Verification items for the finished model (mm, model axes). Face numbers are marked on the shaded views. A direction names the side the tool comes from. Give positions to 0.01 mm unless a question says otherwise; leave off trailing zeros. Write each loop counter-clockwise with the first axis right and the second up, starting at its lowest first coordinate (ties: lowest second). Pieces come first, ordered by that corner, then holes. Notation, with made-up numbers: (12.5, 86.5) - (17.5, 86.5) arc R12 cw to (17.5, 96.5) - close; hole circle Ø7 at (-23, 7). An arc over 180 degrees is marked (long way). Answer as a JSON object with one key per item and string values. Group by question number.
Item 1: Sectioned sample at D-D, the plane z = 9.25. Record the boundary of the cut face in (x, y), and give its area (3 significant figures).
Item 2: Scan lines: line 1 along X through (y, z) = (-12, 6); line 2 along Y through (x, z) = (10, 2.5); line 3 along Z through (x, y) = (0, 6). Record each from-to range of solid material in increasing order. Write a range as [from, to].
Item 3: Sectioned sample at A-A, the plane z = 2.5. Record the boundary of the cut face in (x, y).
Item 4: Go/stop test with flat-tipped pins: pin 1 (5.5 mm diameter, centred on x = -7.5, y = 5.5, fed in from -Z); pin 2 (6.5 mm diameter, centred on x = -10, y = -10, fed in from +Z); pin 3 (1.5 mm diameter, centred on x = -7, z = 8, fed in from +Y); pin 4 (16 mm diameter, centred on x = -10, y = -10, fed in from +Z). Record where each tip stops, or that it passes through.
Item 5: Tool access check on the marked faces 4, 5 and 6. Record the directions out of +Z, -Z, +X, -X, +Y, -Y that give a thin tool (end or side, any length) a straight path to the whole face; none if there is none.
Item 6: Sectioned sample at B-B, the plane y = -10. Record the boundary of the cut face in (x, z), and give its area (3 significant figures).
Item 7: Draft check along X on the marked faces 1, 2 and 3. Enter one of: +X half, -X half, draft (parallel to the pull), parting line (faces both ways), or undercut.
Item 8: Sectioned sample at C-C, the plane x = -6.5. Record the boundary of the cut face in (y, z), and give its area (3 significant figures).
```python
from build123d import *

# Parameters (mm, degrees)
SKETCH_1_W                   = 35
SKETCH_1_H                   = 35
EXTRUDE_1_DEPTH              = 20
CHAMFER_1_SIZE               = 2
M12X1_25_1_D                 = 10.5
HOLE_WIZARD_M8_1_D           = 6.8
HOLE_WIZARD_M5_1_D           = 5.5
HOLE_WIZARD_M5_1_CBORE_D     = 10
HOLE_WIZARD_M5_1_CBORE_DEPTH = 12
SKETCH_11_W                  = 10
SKETCH_11_H                  = 22
CUT_EXTRUDE_1_DEPTH          = 44.945989578


with BuildPart() as part:
    # 草图1 → 凸台-拉伸1 (new body)
    with BuildSketch(Plane.XY):
        Rectangle(SKETCH_1_W, SKETCH_1_H)
    extrude(amount=EXTRUDE_1_DEPTH)

    # 倒角1
    chamfer_1_edges = [part.edges().sort_by_distance(p)[0] for p in [
        (17.5, -17.5, 10),
        (-17.5, -17.5, 10),
        (-17.5, 17.5, 10),
        (17.5, 17.5, 10),
    ]]
    chamfer(chamfer_1_edges, length=CHAMFER_1_SIZE)

    # M12x1.25 螺纹孔1 (through all)
    with Locations(Plane.XY.offset(20)):
        with Locations((7.5, 5.5)):
            Hole(M12X1_25_1_D / 2)

    # M8 螺纹孔1 (through all)
    with Locations(Plane.XY.offset(20)):
        with Locations((-7.5, 5.5)):
            Hole(HOLE_WIZARD_M8_1_D / 2)

    # M5 六角圆柱头螺钉的柱形沉头孔1 (through all)
    with Locations(Plane.XY.offset(20)):
        with Locations((-10, -10), (10, -10)):
            CounterBoreHole(HOLE_WIZARD_M5_1_D / 2, HOLE_WIZARD_M5_1_CBORE_D / 2, HOLE_WIZARD_M5_1_CBORE_DEPTH)

    # 草图11 → 切除-拉伸1 (cut, through all)
    with BuildSketch(Plane(origin=(17.5, 0, 0), x_dir=(0, 0, -1), z_dir=(1, 0, 0))):
        with Locations((-5, 6.5)):
            Rectangle(SKETCH_11_W, SKETCH_11_H)
    extrude(amount=-CUT_EXTRUDE_1_DEPTH, mode=Mode.SUBTRACT)


solid = part.part
```
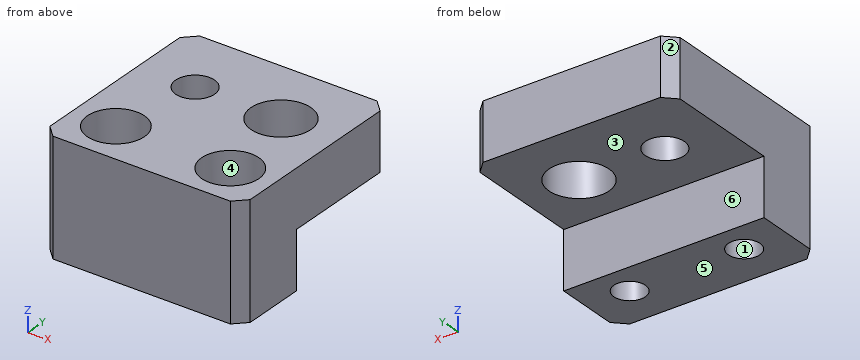
Geometry check:
{
 "1": {"outline": "(-17.5, -15.5) - (-15.5, -17.5) - (15.5, -17.5) - (17.5, -15.5) - (17.5, -4.5) - (-17.5, -4.5) - close; hole circle Ø10 at (-10, -10); hole circle Ø10 at (10, -10)", "area": "294 mm^2"},
 "2": {"line 1": "[-17.5, -11.89], [-8.11, 8.11], [11.89, 17.5]", "line 2": "[-17.5, -12.75], [-7.25, -4.5]", "line 3": "[10, 20]"},
 "3": {"outline": "(-17.5, -15.5) - (-15.5, -17.5) - (15.5, -17.5) - (17.5, -15.5) - (17.5, -4.5) - (-17.5, -4.5) - close; hole circle Ø5.5 at (-10, -10); hole circle Ø5.5 at (10, -10)"},
 "4": {"pin 1": "through", "pin 2": "z = 8", "pin 3": "y = -4.5", "pin 4": "z = 20"},
 "5": {"face 4": "+Z", "face 5": "-Z, +X, -X, +Y, -Y", "face 6": "-Z, +X, -X, +Y"},
 "6": {"outline": "(-17.5, 0) - (-12.75, 0) - (-12.75, 8) - (-15, 8) - (-15, 20) - (-17.5, 20) - close; (-7.25, 0) - (7.25, 0) - (7.25, 8) - (5, 8) - (5, 20) - (-5, 20) - (-5, 8) - (-7.25, 8) - close; (12.75, 0) - (17.5, 0) - (17.5, 20) - (15, 20) - (15, 8) - (12.75, 8) - close", "area": "372 mm^2"},
 "7": {"face 1": "undercut", "face 2": "-X half", "face 3": "draft"},
 "8": {"outline": "(-17.5, 0) - (-4.5, 0) - (-4.5, 10) - (2.25, 10) - (2.25, 20) - (-6.43, 20) - (-6.43, 8) - (-13.57, 8) - (-13.57, 20) - (-17.5, 20) - close; (8.75, 10) - (17.5, 10) - (17.5, 20) - (8.75, 20) - close", "area": "329 mm^2"}
}
